```python
from build123d import *

# Parameters (mm, degrees)
SKETCH1_R           = 5
SKETCH1_R_2         = 3
BOSS_EXTRUDE1_DEPTH = 10
BOSS_EXTRUDE2_START = -10
SKETCH2_R           = 3
BOSS_EXTRUDE2_DEPTH = 10
BOSS_EXTRUDE3_START = -7
BOSS_EXTRUDE3_DEPTH = 4
SKETCH4_W           = 4
SKETCH4_H           = 9.930378158
CUT_EXTRUDE1_DEPTH  = 8
CUT_EXTRUDE3_DEPTH  = 6
SKETCH7_R           = 1
BOSS_EXTRUDE4_DEPTH = 3
SKETCH8_R           = 1.3
BOSS_EXTRUDE5_DEPTH = 1


with BuildPart() as part:
    # Sketch1 → Boss-Extrude1 (new body)
    with BuildSketch(Plane.XY):
        Circle(SKETCH1_R)
        Circle(SKETCH1_R_2, mode=Mode.SUBTRACT)
    extrude(amount=BOSS_EXTRUDE1_DEPTH)

    # Sketch2 → Boss-Extrude2 (add)
    with BuildSketch(Plane.XY.offset(10).offset(BOSS_EXTRUDE2_START)):
        with BuildLine():
            Line((24.88045834, 10.525498272), (14.10478585, 9.738087788))
            add(Edge.make_bspline(
                [(14.10478585, 9.738087788), (8.323441711, 3.769762394), (0, 5)],
                knots=[0, 0, 0, 1, 1, 1], degree=2))
            ThreePointArc((0, 5), (-5, 0), (0, -5))
            add(Edge.make_bspline(
                [(24.88045834, 10.525498272), (16.689881937, -4.631862586), (0, -5)],
                knots=[0, 0, 0, 1, 1, 1], degree=2))
        make_face()
        Circle(SKETCH2_R, mode=Mode.SUBTRACT)
    extrude(amount=BOSS_EXTRUDE2_DEPTH)

    # Sketch3 → Boss-Extrude3 (add)
    with BuildSketch(Plane.XY.offset(10).offset(BOSS_EXTRUDE3_START)):
        with BuildLine():
            Line((-20.423369766, -4.965189079), (0, -4.965189079))
            Line((0, -4.965189079), (0, -3))
            ThreePointArc((0, -3), (-3, 0), (0, 3))
            Line((0, 3), (0, 4.965189079))
            Line((0, 4.965189079), (-20.423369766, 4.965189079))
            Line((-20.423369766, 4.965189079), (-20.423369766, -4.965189079))
        make_face()
    extrude(amount=BOSS_EXTRUDE3_DEPTH)

    # Sketch4 → Cut-Extrude1 (cut)
    with BuildSketch(Plane.ZY.offset(20.423369766)):
        with Locations((5, 0)):
            Rectangle(SKETCH4_W, SKETCH4_H)
    extrude(amount=-CUT_EXTRUDE1_DEPTH, mode=Mode.SUBTRACT)

    # Sketch6 → Cut-Extrude3 (cut)
    with BuildSketch(Plane.XY.offset(7)):
        Polygon((-12.423369766, 1.465189079), (-10.923369766, 1.465189079), (-10.923369766, 2.465189079), (-6.923369766, 2.465189079), (-6.923369766, -2.534810921), (-10.923369766, -2.534810921), (-10.923369766, -1.534810921), (-12.423369766, -1.534810921), align=None)
    extrude(amount=-CUT_EXTRUDE3_DEPTH, mode=Mode.SUBTRACT)

    # Sketch7 → Boss-Extrude4 (add)
    with BuildSketch(Plane.ZY.offset(6.923369766)):
        with Locations(Location((5, 0, 0), (0, 0, 90))):
            Circle(SKETCH7_R)
    extrude(amount=BOSS_EXTRUDE4_DEPTH)

    # Sketch8 → Boss-Extrude5 (add)
    with BuildSketch(Plane.ZY.offset(9.923369766)):
        with Locations(Location((5, 0, 0), (0, 0, 270))):
            Circle(SKETCH8_R)
    extrude(amount=-BOSS_EXTRUDE5_DEPTH)


solid = part.part
```
Build history of the part. All positions in model axes, mm. A direction names the side the tool comes from. Give positions to 0.01 mm unless a question says otherwise; leave off trailing zeros. Order: outer loops, then holes, each group sorted by start corner. A loop starts at its lowest first (then second) coordinate and runs counter-clockwise, first axis right, second up. Notation, with made-up numbers: M -30.75,55.5 L 27.25,55.5 A19 cw 27.25,81.5 Z; hole C 64,-10.75 d6. An arc over 180 degrees is marked long. Return JSON: item names as keys, results as strings.
Q1. Wall check: probe 1 along Y at (x, z) = (-11, 5.5); probe 2 along Y at (x, z) = (0, 5); probe 3 along Z at (x, y) = (-8.5, 4.75). Give the ranges that are in metal, low to high. Write a range as from..to.
Answer list:
{"probe 1": "y = -4.97..-1.53, 1.47..4.97", "probe 2": "y = -5..-3, 3..5", "probe 3": "z = 3..7"}
Q2. 3-axis set-ups, long thin cutter, end or side, ignore diameter. For faces 1 (the face through (-9.43, 0.28, 3.73)), 2 (the face through (-9, -2.535, 5)), 3 (the face through (-12, 1.465, 5)), 4 (the face through (-8, 0, 4)): which of +Z, -Z, +X, -X, +Y, -Y reach the whole face in a straight line?
Answer list:
{"face 1": "-X", "face 2": "+Z, -Z", "face 3": "+Z, -Z, -X", "face 4": "none"}
Q3. Two-plate mould, pull along Y, no slides. Class faces 5 (the face through (-6.6, 0.1, 3)), 6 (the face through (-12, -1.535, 5)), 7 (the face through (-4.966, 0.581, 2.708)): pulls with the +Y half, pulls with the -Y half, needs draft (parallel to the pull), parting line crosses it, or undercut.
Answer list:
{"face 5": "needs draft", "face 6": "undercut", "face 7": "parting line crosses it"}
Q4. Flat gauge pins, fed straight in: pin 1 (1.1 mm diameter, centred on y = -2, z = 4.5, fed in from +X); pin 2 (1 mm diameter, centred on y = 0, z = 7, fed in from +X); pin 3 (0.8 mm diameter, centred on x = -11.5, z = 5.5, fed in from -Y). Where does each tip first touch, or does it go through?
Answer list:
{"pin 1": "stops at x = 13.7", "pin 2": "stops at x = 16.63", "pin 3": "stops at y = -4.97"}
Q5. Band-saw the part on A-A (x = -8). Give the cut face in (y, z), then the cut area to 3 significant figures.
Answer list:
{"outline": "M -4.97,3 L -2.53,3 L -2.53,7 L -4.97,7 Z; C 0,5 d2; M 2.47,3 L 4.97,3 L 4.97,7 L 2.47,7 Z", "area": "22.9 mm^2"}
